from build123d import *

# Parameters (mm, degrees)
SKETCH_1_W      = 208
SKETCH_1_H      = 208
SKETCH_1_W_2    = 200
SKETCH_1_H_2    = 200
EXTRUDE_1_DEPTH = 30


with BuildPart() as part:
    # 草图1 → 拉伸-薄壁1 (new body)
    with BuildSketch(Plane.XY):
        Rectangle(SKETCH_1_W, SKETCH_1_H)
        Rectangle(SKETCH_1_W_2, SKETCH_1_H_2, mode=Mode.SUBTRACT)
    extrude(amount=EXTRUDE_1_DEPTH)


solid = part.part
Source: CAD feature listing. Evaluate the final solid. Frame: model axes, mm. A direction names the side the tool comes from. Give positions to 0.01 mm unless a question says otherwise; leave off trailing zeros. Loops run counter-clockwise (first coordinate to the right, second up) from the corner with the lowest first, then second, coordinate; pieces in that order, holes last. Notation, with made-up numbers: (-6.5, 23) -> (14.5, 23) arc R15 cw to (14.5, 42) -> close; hole circle Ø3 at (79.25, -31). An arc over 180 degrees is marked (long way). Use a Markdown table: item, result. Add a question column.
1) Section query C-C, the plane z = 27.25. Return the cut outline in (x, y), then the cut area to 3 significant figures.
2) Line query: line 1 along X through (y, z) = (48, 19.25). Output: solid intervals per line, ascending. Write a range as [from, to].
3) Section query A-A, the plane x = -1. Return the cut outline in (y, z).
4) Reachability of faces 1 (the face through (-101, 47, 0)), 2 (the face through (-100, -1, 15)) from +Z, -Z, +X, -X, +Y, -Y: full face, straight path, thin tool, end or side. Return the list, or none.
5) Pull-direction query (X, two-part tool) for faces 3 (the face through (100, -1, 15)), 4 (the face through (-104, -1, 15)), 5 (the face through (-1, -104, 15)); classes: +X half, -X half, draft (parallel to the pull), parting line (faces both ways), or undercut.
Numbers:
| question | item | result |
|---|---|---|
| 1 | outline | (-104, -104) -> (104, -104) -> (104, 104) -> (-104, 104) -> close; hole (-100, -100) -> (100, -100) -> (100, 100) -> (-100, 100) -> close |
| 1 | area | 3,260 mm2 |
| 2 | line 1 | x = [-104, -100], [100, 104] |
| 3 | outline | (-104, 0) -> (-100, 0) -> (-100, 30) -> (-104, 30) -> close; (100, 0) -> (104, 0) -> (104, 30) -> (100, 30) -> close |
| 4 | face 1 | -Z, +X, -X, +Y, -Y |
| 4 | face 2 | +Z, -Z |
| 5 | face 3 | undercut |
| 5 | face 4 | -X half |
| 5 | face 5 | draft |
